Geometry check sheet. Reference: the model listing, model coordinates, mm. A direction names the side the tool comes from. Coordinates: 2 decimals unless noted, no trailing zeros. Loops run counter-clockwise (first coordinate to the right, second up) from the corner with the lowest first, then second, coordinate; pieces in that order, holes last.
from build123d import *

# Parameters (mm, degrees)
SKETCH1_R           = 5.25
SKETCH1_R_2         = 0.5
BOSS_EXTRUDE1_DEPTH = 3


with BuildPart() as part:
    # Sketch1 → Boss-Extrude1 (new body)
    with BuildSketch(Plane.XY):
        with BuildLine():
            Line((86, 0), (86, 3))
            Line((86, 3), (78, 3))
            ThreePointArc((78, 3), (76.585786438, 3.585786438), (76, 5))
            Line((76, 5), (76, 46))
            ThreePointArc((76, 46), (74.535533906, 49.535533906), (71, 51))
            Line((71, 51), (15, 51))
            ThreePointArc((15, 51), (11.464466094, 49.535533906), (10, 46))
            Line((10, 46), (10, 5))
            ThreePointArc((10, 5), (9.414213562, 3.585786438), (8, 3))
            Line((8, 3), (0, 3))
            Line((0, 3), (0, 0))
            Line((0, 0), (86, 0))
        make_face()
        with Locations((43, 20)):
            Circle(SKETCH1_R, mode=Mode.SUBTRACT)
        with Locations((25, 50)):
            Circle(SKETCH1_R_2, mode=Mode.SUBTRACT)
        with Locations((61, 50)):
            Circle(SKETCH1_R_2, mode=Mode.SUBTRACT)
        with Locations((75, 25)):
            Circle(SKETCH1_R_2, mode=Mode.SUBTRACT)
        with Locations((11, 25)):
            Circle(SKETCH1_R_2, mode=Mode.SUBTRACT)
    extrude(amount=BOSS_EXTRUDE1_DEPTH)


solid = part.part
(1) Sectioned sample at C-C on z = 0.9. Record the cut outline in (x, y).
Findings:
outline: (0, 0) - (86, 0) - (86, 3) - (78, 3) arc R2 cw to (76, 5) - (76, 46) arc R5 ccw to (71, 51) - (15, 51) arc R5 ccw to (10, 46) - (10, 5) arc R2 cw to (8, 3) - (0, 3) - close; hole circle Ø1 at (11, 25); hole circle Ø1 at (25, 50); hole circle Ø10.5 at (43, 20); hole circle Ø1 at (61, 50); hole circle Ø1 at (75, 25)
(2) Sectioned sample at D-D on x = 80.5. Record the cut outline in (y, z).
Findings:
outline: (0, 0) - (3, 0) - (3, 3) - (0, 3) - close
(3) Sectioned sample at B-B on y = 20. Record the cut outline in (x, z).
Findings:
outline: (10, 0) - (37.75, 0) - (37.75, 3) - (10, 3) - close; (48.25, 0) - (76, 0) - (76, 3) - (48.25, 3) - close
(4) Access from +Z, -Z, +X, -X, +Y, -Y to the whole of each face (thin tool, end or side, straight path). Record for faces 4 (the flat face through (10, 26, 1)), 5 (the flat face through (82, 3, 1)), 6 (the flat face through (42, 26, 3)).
Findings:
face 4: +Z, -Z, -X, +Y
face 5: +Z, -Z, +X, +Y
face 6: +Z, +X, -X, +Y, -Y
(5) Gauge pin test, flat ends, axial feed: pin 1 Ø1 at (y, z) = (33, 1) entering from +X; pin 2 Ø1.5 at (y, z) = (23, 1.5) entering from -X. Record the tip position at first contact, or that the pin passes through.
Findings:
pin 1: stops at x = 76
pin 2: stops at x = 10
(6) Scan lines: L1, parallel to Y at x = 25, z = 0.75; L2, parallel to Y at x = 43, z = 1.2; L3, parallel to X at y = 50, z = 2.05. Record each from-to range of solid material in increasing order.
Findings:
L1: y = 0 to 49.5, 50.5 to 51
L2: y = 0 to 14.75, 25.25 to 51
L3: x = 12 to 24.5, 25.5 to 60.5, 61.5 to 74
(7) Draft check along Y on faces 1 (the flat face through (86, 1, 1)), 2 (the cylindrical face through (38.83, 16.81, 1.48)), 3 (the cylindrical face through (76.6, 3.57, 1.48)). Enter one of: +Y half, -Y half, draft (parallel to the pull), parting line (faces both ways), or undercut.
Findings:
face 1: draft
face 2: undercut
face 3: +Y half
(8) Sectioned sample at A-A on x = 43. Record the cut outline in (y, z), and give its area (4 significant figures).
Findings:
outline: (0, 0) - (14.75, 0) - (14.75, 3) - (0, 3) - close; (25.25, 0) - (51, 0) - (51, 3) - (25.25, 3) - close
area: 121.5 mm2
